Verification items for the finished model (mm, model axes). Give positions to 0.01 mm unless a question says otherwise; leave off trailing zeros. Write each loop counter-clockwise with the first axis right and the second up, starting at its lowest first coordinate (ties: lowest second). Pieces come first, ordered by that corner, then holes. Notation, with made-up numbers: (50.5, 7) -> (74.5, 7) arc R26 ccw to (74.5, 41) -> close; hole circle Ø2 at (25, 28). An arc over 180 degrees is marked (long way). Write item = value, one per line.
from build123d import *

# Parameters (mm, degrees)
EXTRUDE_1_DEPTH           = 40
SKETCH_2_R                = 20
CUT_EXTRUDE_1_DEPTH       = 10
HOLE_WIZARD_0_D           = 15.5
HOLE_WIZARD_0_CBORE_D     = 24
HOLE_WIZARD_0_CBORE_DEPTH = 15
SKETCH_5_R                = 47.5
CUT_EXTRUDE_2_DEPTH       = 911.7848264
SKETCH_6_R                = 32.5
CUT_EXTRUDE_3_DEPTH       = 911.7848264
FILLET_1_R                = 20


with BuildPart() as part:
    # 草图1 → 凸台-拉伸1 (new body)
    with BuildSketch(Plane(origin=(0, 0, 0), x_dir=(1, 0, 0), z_dir=(0, 1, 0))):
        Polygon((-480, 480), (480, 480), (480, 152.5), (773, 152.5), (773, -152.5), (480, -152.5), (480, -480), (-480, -480), (-480, -152.5), (-773, -152.5), (-773, 152.5), (-480, 152.5), align=None)
    extrude(amount=EXTRUDE_1_DEPTH)

    # 草图2 → 切除-拉伸1 (cut)
    with BuildSketch(Plane.XZ):
        with Locations(Location((602.5, 0, 0), (0, 0, 270))):
            Circle(SKETCH_2_R)
    cut_extrude_1 = extrude(amount=-CUT_EXTRUDE_1_DEPTH, mode=Mode.SUBTRACT)

    # 打孔尺寸(%根据)内六角圆柱头螺钉的类型0 (through all)
    with Locations(Plane(origin=(0, 40, 0), x_dir=(1, 0, 0), z_dir=(0, 1, 0))):
        with Locations((602.5, 0)):
            hole_wizard_0 = CounterBoreHole(HOLE_WIZARD_0_D / 2, HOLE_WIZARD_0_CBORE_D / 2, HOLE_WIZARD_0_CBORE_DEPTH)

    # 镜向1: 切除-拉伸1, 打孔尺寸(%根据)内六角圆柱头螺钉的类型0 across plane
    add(cut_extrude_1.mirror(Plane(origin=(0, 0, 0), x_dir=(0, 0, 1), z_dir=(1, 0, 0))), mode=Mode.SUBTRACT)
    add(hole_wizard_0.mirror(Plane(origin=(0, 0, 0), x_dir=(0, 0, 1), z_dir=(1, 0, 0))), mode=Mode.SUBTRACT)

    # 草图5 → 切除-拉伸2 (cut, through all)
    with BuildSketch(Plane.XZ):
        with Locations(Location((490, 0, 0), (0, 0, 270))):
            Circle(SKETCH_5_R)
    cut_extrude_2 = extrude(amount=-CUT_EXTRUDE_2_DEPTH, mode=Mode.SUBTRACT)

    # 镜向2: 切除-拉伸2 across plane
    add(cut_extrude_2.mirror(Plane(origin=(0, 0, 0), x_dir=(0, 0, 1), z_dir=(1, 0, 0))), mode=Mode.SUBTRACT)

    # 草图6 → 切除-拉伸3 (cut, through all)
    with BuildSketch(Plane(origin=(0, 40, 0), x_dir=(1, 0, 0), z_dir=(0, 1, 0))):
        with Locations(Location((0, 0, 0), (0, 0, 270))):
            Circle(SKETCH_6_R)
    extrude(amount=-CUT_EXTRUDE_3_DEPTH, mode=Mode.SUBTRACT)

    # 圆角1
    fillet_1_edges = [part.edges().sort_by_distance(p)[0] for p in [
        (-480, 20, 152.5),
        (-480, 20, -152.5),
        (480, 20, -152.5),
        (480, 20, 152.5),
    ]]
    fillet(fillet_1_edges, radius=FILLET_1_R)


solid = part.part
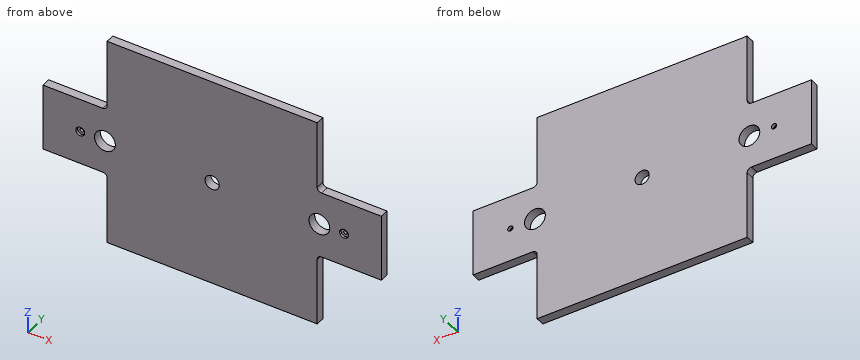
Item 1: Go/stop test with flat-tipped pins: P1, Ø12, axis at x = -606, y = 28.5, coming from the +Z side; P2, Ø3, axis at y = 31, z = -170, coming from the +X side; P3, Ø3, axis at y = 10, z = 192, coming from the -X side; P4, Ø9.5, axis at x = -602.5, z = 0, coming from the -Y side. Record where each tip stops, or that it passes through.
Response values:
P1 = 152.5
P2 = 480.4
P3 = -480
P4 = through
Item 2: Material ranges on line 1 (X direction, y = 9, z = 0); line 2 (Z direction, x = -602.5, y = 14); line 3 (X direction, y = 29, z = 218), recorded low to high.
Response values:
line_1 = -773 to -622.5, -582.5 to -537.5, -442.5 to -32.5, 32.5 to 442.5, 537.5 to 582.5, 622.5 to 773
line_2 = -152.5 to -7.75, 7.75 to 152.5
line_3 = -480 to 480
Item 3: Sectioned sample at A-A on z = 354. Record the cut outline in (x, y), then the cut area to 3 significant figures.
Response values:
outline = (-480, 0) -> (480, 0) -> (480, 40) -> (-480, 40) -> close
area = 38,400 mm^2
